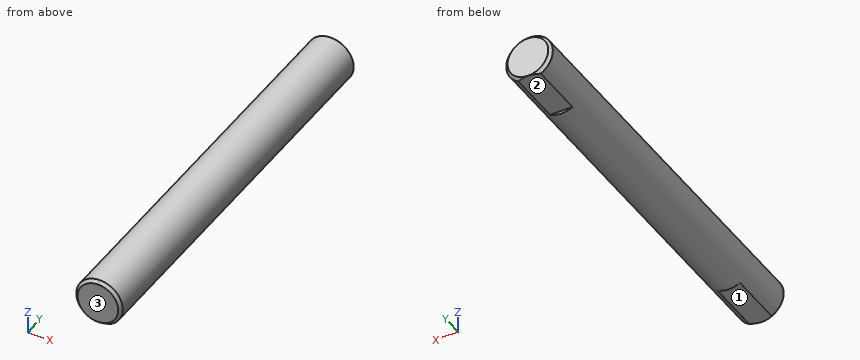
from build123d import *
from build123d.topology import SkipClean

# Parameters (mm, degrees)
SKETCH1_R           = 4
BOSS_EXTRUDE1_DEPTH = 70
CHAMFER1_SIZE       = 0.5
SKETCH2_W           = 1.564608121
SKETCH2_H           = 10
CUT_EXTRUDE1_DEPTH  = 5


with BuildPart() as part:
    # Sketch1 → Boss-Extrude1 (new body)
    with BuildSketch(Plane(origin=(0, 0, 0), x_dir=(1, 0, 0), z_dir=(0, 1, 0))):
        with Locations(Location((0, 0, 0), (0, 0, 270))):
            Circle(SKETCH1_R)
    extrude(amount=BOSS_EXTRUDE1_DEPTH)

    # Chamfer1
    chamfer1_edges = [part.edges().sort_by_distance(p)[0] for p in [
        (0, 0, -4),
        (0, 70, -4),
    ]]
    chamfer(chamfer1_edges, length=CHAMFER1_SIZE)

    # Sketch2 → Cut-Extrude1 (cut, symmetric)
    with SkipClean():  # the faces are left unmerged after this step: merging them gives an invalid solid
        with BuildSketch(Plane(origin=(0, 0, 0), x_dir=(0, 0, -1), z_dir=(1, 0, 0))):
            with Locations((4.28230406, 65)):
                Rectangle(SKETCH2_W, SKETCH2_H)
            with Locations((4.28230406, 5)):
                Rectangle(SKETCH2_W, SKETCH2_H)
        extrude(amount=CUT_EXTRUDE1_DEPTH, both=True, mode=Mode.SUBTRACT)


solid = part.part
Work out the finished part from the listing and answer in its coordinate system (mm). Face numbers are marked on the shaded views. A direction names the side the tool comes from. Round coordinates to 2 decimals unless told otherwise and drop trailing zeros. Loops run counter-clockwise (first coordinate to the right, second up) from the corner with the lowest first, then second, coordinate; pieces in that order, holes last. Notation, with made-up numbers: M 29.25,68 L 46.25,68 A23 ccw 46.25,78 Z; hole C 16.25,-6.75 d10. An arc over 180 degrees is marked long. One line per question, with ' | ' between items. Start each with the question number.
(1) A cutting plane is placed at A-A on y = 23.5. Write down the section's boundary in (x, z).
(2) A tool of negligible diameter and unlimited length cuts with its end or side. For the marked faces 1, 2 and 3, from which of +Z, -Z, +X, -X, +Y, -Y can it reach the whole face along a straight path? Write none if from no direction.
(3) Flat-ended cylindrical pins translate along their axes: pin 1 Ø0.6 at (x, z) = (1, -4) entering from -Y; pin 2 Ø1.9 at (x, y) = (-1, 66.5) entering from -Z; pin 3 Ø3 at (y, z) = (21, 2.5) entering from -X. Find the tip coordinate at first contact, or state that the pin passes through.
(4) Find the intervals of material crossed by line 1 (X direction, y = 61, z = 3.5); line 2 (Z direction, x = -2.75, y = 44.5), in increasing order.
Geometry check:
1) outline: C 0,0 d8
2) face 1: -Z, +X, -X, -Y | face 2: -Z, +X, -X, +Y | face 3: +Z, -Z, +X, -X, -Y
3) pin 1: stops at y = 10 | pin 2: stops at z = -3.5 | pin 3: stops at x = -3.87
4) line 1: x = -1.94 to 1.94 | line 2: z = -2.9 to 2.9
